```python
from build123d import *

# Parameters (mm, degrees)
SKETCH_1_W                = 160
SKETCH_1_H                = 300
EXTRUDE_1_DEPTH           = 20
HOLE_WIZARD_1_D           = 15.5
HOLE_WIZARD_1_DEPTH       = 25
HOLE_WIZARD_1_CBORE_D     = 24
HOLE_WIZARD_1_CBORE_DEPTH = 15
HOLE_WIZARD_1_TIP         = 4.656669797
CHAMFER_1_SIZE            = 5
HOLE_WIZARD_0_D           = 6.6
HOLE_WIZARD_0_DEPTH       = 25
HOLE_WIZARD_0_CBORE_D     = 11
HOLE_WIZARD_0_CBORE_DEPTH = 6.8
HOLE_WIZARD_0_TIP         = 1.982840043
SKETCH_6_R                = 8.1
SKETCH_6_R_2              = 10
CUT_EXTRUDE_1_DEPTH       = 2
HOLE_WIZARD_M5_1_D        = 4.2
HOLE_WIZARD_M5_1_DEPTH    = 20
HOLE_WIZARD_M5_1_TIP      = 1.2618073
HOLE_WIZARD_M5_2_D        = 4.2
HOLE_WIZARD_M5_2_DEPTH    = 20
HOLE_WIZARD_M5_2_TIP      = 1.2618073
HOLE_WIZARD_M5_3_D        = 4.2
HOLE_WIZARD_M5_3_DEPTH    = 25
HOLE_WIZARD_M5_3_TIP      = 1.2618073


with BuildPart() as part:
    # 草图1 → 凸台-拉伸1 (new body)
    with BuildSketch(Plane(origin=(0, 0, 0), x_dir=(0, 0, -1), z_dir=(1, 0, 0))):
        Rectangle(SKETCH_1_W, SKETCH_1_H)
    extrude(amount=EXTRUDE_1_DEPTH)

    # 打孔尺寸(%根据)内六角圆柱头螺钉的类型1
    with Locations(Plane(origin=(20, 0, 0), x_dir=(0, 0, -1), z_dir=(1, 0, 0))):
        with Locations((0, 25)):
            CounterBoreHole(HOLE_WIZARD_1_D / 2, HOLE_WIZARD_1_CBORE_D / 2, HOLE_WIZARD_1_CBORE_DEPTH, depth=HOLE_WIZARD_1_DEPTH)
            with Locations((0, 0, -(HOLE_WIZARD_1_DEPTH + HOLE_WIZARD_1_TIP / 2))):  # 118° drill point
                Cone(0, HOLE_WIZARD_1_D / 2, HOLE_WIZARD_1_TIP, mode=Mode.SUBTRACT)

    # 倒角1
    chamfer_1_edges = [part.edges().sort_by_distance(p)[0] for p in [
        (10, -150, -80),
        (10, -150, 80),
        (10, 150, 80),
        (10, 150, -80),
    ]]
    chamfer(chamfer_1_edges, length=CHAMFER_1_SIZE)

    # 打孔尺寸(%根据)内六角圆柱头螺钉的类型0
    with Locations(Plane(origin=(20, 0, 0), x_dir=(0, 0, -1), z_dir=(1, 0, 0))):
        with Locations((40, -30), (40, 80), (-40, -30), (-40, 80)):
            CounterBoreHole(HOLE_WIZARD_0_D / 2, HOLE_WIZARD_0_CBORE_D / 2, HOLE_WIZARD_0_CBORE_DEPTH, depth=HOLE_WIZARD_0_DEPTH)
            with Locations((0, 0, -(HOLE_WIZARD_0_DEPTH + HOLE_WIZARD_0_TIP / 2))):  # 118° drill point
                Cone(0, HOLE_WIZARD_0_D / 2, HOLE_WIZARD_0_TIP, mode=Mode.SUBTRACT)

    # 草图6 → 切除-拉伸1 (cut)
    with BuildSketch(Plane.ZY):
        with Locations((-40, 80)):
            Circle(SKETCH_6_R)
        with Locations((-40, -30)):
            Circle(SKETCH_6_R)
        with Locations((0, 25)):
            Circle(SKETCH_6_R_2)
        with Locations((40, -30)):
            Circle(SKETCH_6_R)
        with Locations((40, 80)):
            Circle(SKETCH_6_R)
    extrude(amount=-CUT_EXTRUDE_1_DEPTH, mode=Mode.SUBTRACT)

    # M5 螺纹孔1
    with Locations(Plane.ZY):
        with Locations((65, -96), (35, -96), (65, 4), (35, 4), (65, 104), (35, 104), (-35, 104), (-65, 104), (-35, 4), (-65, 4), (-35, -96), (-65, -96)):
            Hole(HOLE_WIZARD_M5_1_D / 2, depth=HOLE_WIZARD_M5_1_DEPTH)
            with Locations((0, 0, -(HOLE_WIZARD_M5_1_DEPTH + HOLE_WIZARD_M5_1_TIP / 2))):  # 118° drill point
                Cone(0, HOLE_WIZARD_M5_1_D / 2, HOLE_WIZARD_M5_1_TIP, mode=Mode.SUBTRACT)

    # M5 螺纹孔2
    with Locations(Plane.ZY):
        with Locations((72.5, -143), (72.5, -128)):
            Hole(HOLE_WIZARD_M5_2_D / 2, depth=HOLE_WIZARD_M5_2_DEPTH)
            with Locations((0, 0, -(HOLE_WIZARD_M5_2_DEPTH + HOLE_WIZARD_M5_2_TIP / 2))):  # 118° drill point
                Cone(0, HOLE_WIZARD_M5_2_D / 2, HOLE_WIZARD_M5_2_TIP, mode=Mode.SUBTRACT)

    # M5 螺纹孔3
    with Locations(Plane.ZY):
        with Locations((-73.5, -143), (-73.5, -128)):
            Hole(HOLE_WIZARD_M5_3_D / 2, depth=HOLE_WIZARD_M5_3_DEPTH)
            with Locations((0, 0, -(HOLE_WIZARD_M5_3_DEPTH + HOLE_WIZARD_M5_3_TIP / 2))):  # 118° drill point
                Cone(0, HOLE_WIZARD_M5_3_D / 2, HOLE_WIZARD_M5_3_TIP, mode=Mode.SUBTRACT)


solid = part.part
```
Verification items for the finished model (mm, model axes). A direction names the side the tool comes from. Give positions to 0.01 mm unless a question says otherwise; leave off trailing zeros. Order: outer loops, then holes, each group sorted by start corner. A loop starts at its lowest first (then second) coordinate and runs counter-clockwise, first axis right, second up. Notation, with made-up numbers: (7.25, -28.75) -> (20.25, -28.75) arc R26 cw to (20.25, -6.75) -> close; hole circle Ø7 at (2, 28). An arc over 180 degrees is marked (long way). Use a Markdown table: item, result.
1) Material ranges on probe 1 along Y at (x, z) = (13, -35); probe 2 along Z at (x, y) = (5.75, 104); probe 3 along Y at (x, z) = (12, 72.5), recorded low to high.
Results:
| item | result |
|---|---|
| probe 1 | -150 to -98.1, -93.9 to 1.9, 6.1 to 101.9, 106.1 to 150 |
| probe 2 | -80 to -67.1, -62.9 to -37.1, -32.9 to 32.9, 37.1 to 62.9, 67.1 to 80 |
| probe 3 | -150 to -145.1, -140.9 to -130.1, -125.9 to 150 |
2) Section check D-D, the plane z = 1. Record the boundary of the cut face in (x, y).
Results:
| item | result |
|---|---|
| outline | (0, -150) -> (20, -150) -> (20, 13.04) -> (5, 13.04) -> (5, 17.31) -> (2, 17.31) -> (2, 15.05) -> (0, 15.05) -> close; (0, 34.95) -> (2, 34.95) -> (2, 32.69) -> (5, 32.69) -> (5, 36.96) -> (20, 36.96) -> (20, 150) -> (0, 150) -> close |
3) Section check A-A, the plane z = 40. Record the boundary of the cut face in (x, y).
Results:
| item | result |
|---|---|
| outline | (0, -150) -> (20, -150) -> (20, -35.5) -> (13.2, -35.5) -> (13.2, -33.3) -> (2, -33.3) -> (2, -38.1) -> (0, -38.1) -> close; (0, -21.9) -> (2, -21.9) -> (2, -26.7) -> (13.2, -26.7) -> (13.2, -24.5) -> (20, -24.5) -> (20, 74.5) -> (13.2, 74.5) -> (13.2, 76.7) -> (2, 76.7) -> (2, 71.9) -> (0, 71.9) -> close; (0, 88.1) -> (2, 88.1) -> (2, 83.3) -> (13.2, 83.3) -> (13.2, 85.5) -> (20, 85.5) -> (20, 150) -> (0, 150) -> close |
4) Section check B-B, the plane x = 17.25. Give the number of separate pieces and of enclosed holes in the cut face, then the cut area to 3 significant figures.
Results:
| item | result |
|---|---|
| separate pieces | 1 |
| enclosed holes | 21 |
| area | 46,900 mm² |
5) Depth check by flat-ended pin: pin 1 Ø12.5 at (y, z) = (-30, -40) entering from -X; pin 2 Ø9.5 at (y, z) = (80, -40) entering from +X; pin 3 Ø7 at (y, z) = (29, -2) entering from +X. Enter the tip coordinate at first touch or a pass-through.
Results:
| item | result |
|---|---|
| pin 1 | x = 2 |
| pin 2 | x = 13.2 |
| pin 3 | x = 5 |
6) Section check C-C, the plane y = 25. Record the boundary of the cut face in (x, z), then the cut area to 3 significant figures.
Results:
| item | result |
|---|---|
| outline | (0, -80) -> (20, -80) -> (20, -12) -> (5, -12) -> (5, -7.75) -> (2, -7.75) -> (2, -10) -> (0, -10) -> close; (0, 10) -> (2, 10) -> (2, 7.75) -> (5, 7.75) -> (5, 12) -> (20, 12) -> (20, 80) -> (0, 80) -> close |
| area | 2,750 mm² |
7) Mould release check, pull along Y, two halves, no side actions. Record for faces 1 (the flat face through (10, -2, 80)), 2 (the cylindrical face through (7.52, -27.77, 37.57)), 3 (the flat face through (10, -150, 1)): pulls with the +Y half, pulls with the -Y half, needs draft (parallel to the pull), parting line crosses it, or undercut.
Results:
| item | result |
|---|---|
| face 1 | needs draft |
| face 2 | undercut |
| face 3 | pulls with the -Y half |
8) Tool access check on faces 4 (the flat face through (2, 76.5, 39.9)), 5 (the flat face through (5, 25, -8)), 6 (the flat face through (10, 150, 1)). Record the directions out of +Z, -Z, +X, -X, +Y, -Y that give a thin tool (end or side, any length) a straight path to the whole face; none if there is none.
Results:
| item | result |
|---|---|
| face 4 | -X |
| face 5 | +X |
| face 6 | +Z, -Z, +X, -X, +Y |
